Part model, mm, in its own coordinate system. A direction names the side the tool comes from. Round coordinates to 2 decimals unless told otherwise and drop trailing zeros. Write each loop counter-clockwise with the first axis right and the second up, starting at its lowest first coordinate (ties: lowest second). Pieces come first, ordered by that corner, then holes.
```python
from build123d import *

# Parameters (mm, degrees)
SKETCH1_R               = 465
SKETCH1_R_2             = 225
BOSS_EXTRUDE1_DEPTH     = 30
SKETCH2_R               = 308
CUT_EXTRUDE1_DEPTH      = 5
CUT_EXTRUDE7_DEPTH      = 659.293247725
CUT_EXTRUDE7_DEPTH_BACK = 659.293247725
SKETCH4_R               = 11


with BuildPart() as part:
    # Sketch1 → Boss-Extrude1 (new body)
    with BuildSketch(Plane.XY):
        Circle(SKETCH1_R)
        Circle(SKETCH1_R_2, mode=Mode.SUBTRACT)
    extrude(amount=BOSS_EXTRUDE1_DEPTH)

    # Sketch2 → Cut-Extrude1 (cut)
    with BuildSketch(Plane.XY.offset(30)):
        Circle(SKETCH2_R)
    extrude(amount=-CUT_EXTRUDE1_DEPTH, mode=Mode.SUBTRACT)

    # Sketch4 → Cut-Extrude7 (cut, two sides: drawn at the far end of the back side and taken through both)
    with BuildSketch(Plane(origin=(0, 0, 0), x_dir=(-1, 0, 0), z_dir=(0, 0, -1)).offset(-CUT_EXTRUDE7_DEPTH_BACK)):
        with Locations(Location((-260.799973098, 69.881142178, 0), (0, 0, 180))):
            Circle(SKETCH4_R)
        with Locations(Location((-190.91883092, 190.91883092, 0), (0, 0, 180))):
            Circle(SKETCH4_R)
        with Locations(Location((-69.881142178, 260.799973098, 0), (0, 0, 180))):
            Circle(SKETCH4_R)
        with Locations(Location((69.881142178, 260.799973098, 0), (0, 0, 180))):
            Circle(SKETCH4_R)
        with Locations(Location((190.91883092, 190.91883092, 0), (0, 0, 180))):
            Circle(SKETCH4_R)
        with Locations(Location((260.799973098, 69.881142178, 0), (0, 0, 180))):
            Circle(SKETCH4_R)
        with Locations(Location((260.799973098, -69.881142178, 0), (0, 0, 180))):
            Circle(SKETCH4_R)
        with Locations(Location((190.91883092, -190.91883092, 0), (0, 0, 180))):
            Circle(SKETCH4_R)
        with Locations(Location((69.881142178, -260.799973098, 0), (0, 0, 180))):
            Circle(SKETCH4_R)
        with Locations(Location((-69.881142178, -260.799973098, 0), (0, 0, 180))):
            Circle(SKETCH4_R)
        with Locations(Location((-190.91883092, -190.91883092, 0), (0, 0, 180))):
            Circle(SKETCH4_R)
        with Locations(Location((-260.799973098, -69.881142178, 0), (0, 0, 180))):
            Circle(SKETCH4_R)
    extrude(amount=CUT_EXTRUDE7_DEPTH + CUT_EXTRUDE7_DEPTH_BACK, mode=Mode.SUBTRACT)


solid = part.part
```
Q1. Cut at C-C on z = 6. State how many separate pieces and enclosed holes the cut face has, plus the area to 3 significant figures.
Values follow:
separate pieces: 1
enclosed holes: 13
area: 516,000 mm2
Q2. Wall check: L1, parallel to X at y = 255, z = 23; L2, parallel to X at y = -77, z = 5; L3, parallel to Y at x = 60.5, z = 21. Give the ranges that are in metal, low to high.
Values follow:
L1: x = -388.84 to -79.23, -60.53 to 60.53, 79.23 to 388.84
L2: x = -458.58 to -269.19, -252.41 to -211.41, 211.41 to 252.41, 269.19 to 458.58
L3: y = -461.05 to -266.54, -255.06 to -216.71, 216.71 to 255.06, 266.54 to 461.05
Q3. Which spindle directions (+Z, -Z, +X, -X, +Y, -Y) get a long thin tool onto all of the face, cutting with end or side? Do faces 1 (the cylindrical face through (271.3, 66.6, 12.7)), 2 (the flat face through (90, 207, 25)). Say none if no direction does.
Values follow:
face 1: +Z, -Z
face 2: +Z
Q4. Cut at A-A on x = 0. Write the cut outline in (y, z).
Values follow:
outline: (-465, 0) - (-225, 0) - (-225, 25) - (-308, 25) - (-308, 30) - (-465, 30) - close; (225, 0) - (465, 0) - (465, 30) - (308, 30) - (308, 25) - (225, 25) - close
Q5. Cut at D-D on y = -287. Write the cut outline in (x, z).
Values follow:
outline: (-365.86, 0) - (365.86, 0) - (365.86, 30) - (111.78, 30) - (111.78, 25) - (-111.78, 25) - (-111.78, 30) - (-365.86, 30) - close
Q6. Drop flat-ended pins along their axis: pin 1 (12 mm diameter, centred on x = 289.5, z = 22.5, fed in from +Y); pin 2 (17.5 mm diameter, centred on x = -69.88, y = -260.8, fed in from -Z); pin 3 (2 mm diameter, centred on x = 281.5, z = 25, fed in from +Y); pin 4 (1.5 mm diameter, centred on x = 182.5, z = 13.5, fed in from +Y). Give the stop position or say it passes through.
Values follow:
pin 1: stops at y = 368.58
pin 2: passes through
pin 3: stops at y = 370.87
pin 4: stops at y = 428.01
Q7. Mould opens along X. For faces 3 (the cylindrical face through (-369.008, -282.945, 14.79)), 4 (the cylindrical face through (-201.91, 190.44, 12.67)), 5 (the flat face through (200, 110, 0)), 6 (the cylindrical face through (-244.42, -187.41, 27.54)) say: +X half, -X half, draft (parallel to the pull), parting line (faces both ways), or undercut.
Values follow:
face 3: parting line
face 4: undercut
face 5: draft
face 6: undercut
